from build123d import *

# Parameters (mm, degrees)
SKETCH1_W           = 40
SKETCH1_H           = 40
SKETCH1_W_2         = 36
SKETCH1_H_2         = 36
BOSS_EXTRUDE1_DEPTH = 1116
FILLET1_R           = 2
FILLET2_R           = 4


with BuildPart() as part:
    # Sketch1 → Boss-Extrude1 (new body)
    with BuildSketch(Plane.XY):
        Rectangle(SKETCH1_W, SKETCH1_H)
        Rectangle(SKETCH1_W_2, SKETCH1_H_2, mode=Mode.SUBTRACT)
    extrude(amount=BOSS_EXTRUDE1_DEPTH)

    # Fillet1
    fillet1_edges = [part.edges().sort_by_distance(p)[0] for p in [
        (18, -18, 558),
        (18, 18, 558),
        (-18, 18, 558),
        (-18, -18, 558),
    ]]
    fillet(fillet1_edges, radius=FILLET1_R)

    # Fillet2
    fillet2_edges = [part.edges().sort_by_distance(p)[0] for p in [
        (20, -20, 558),
        (-20, -20, 558),
        (-20, 20, 558),
        (20, 20, 558),
    ]]
    fillet(fillet2_edges, radius=FILLET2_R)


solid = part.part
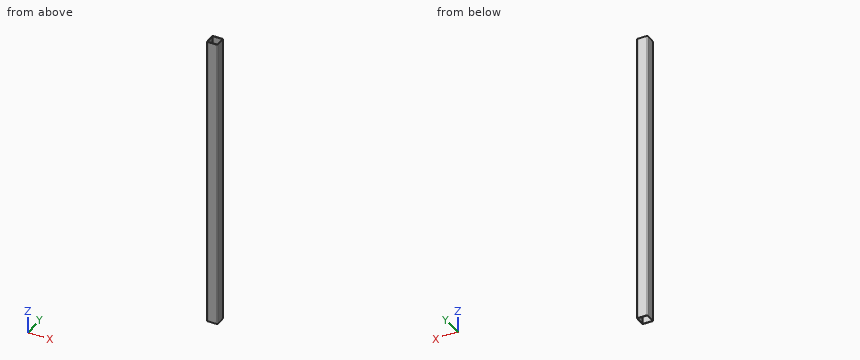
Verification items for the finished model (mm, model axes). Coordinates: 2 decimals unless noted, no trailing zeros. Write each loop counter-clockwise with the first axis right and the second up, starting at its lowest first coordinate (ties: lowest second). Pieces come first, ordered by that corner, then holes. Notation, with made-up numbers: M -22,-23 L 35,-23 A20 ccw 35,-3 Z; hole C 51.5,10.5 d4. An arc over 180 degrees is marked long. Use a Markdown table: item, result.
Q1. Sectioned sample at C-C, the plane z = 978. Record the boundary of the cut face in (x, y).
Reply:
| item | result |
|---|---|
| outline | M -20,-16 A4 ccw -16,-20 L 16,-20 A4 ccw 20,-16 L 20,16 A4 ccw 16,20 L -16,20 A4 ccw -20,16 Z; hole M -18,-16 A2 ccw -16,-18 L 16,-18 A2 ccw 18,-16 L 18,16 A2 ccw 16,18 L -16,18 A2 ccw -18,16 Z |
Q2. Sectioned sample at A-A, the plane x = -6.5. Record the boundary of the cut face in (y, z).
Reply:
| item | result |
|---|---|
| outline | M -20,0 L -18,0 L -18,1116 L -20,1116 Z; M 18,0 L 20,0 L 20,1116 L 18,1116 Z |
Q3. Thickness scan on line 1 (Y direction, x = 10, z = 511.5); line 2 (Y direction, x = -17.5, z = 381.5). Record the ranges inside material, lowest first.
Reply:
| item | result |
|---|---|
| line 1 | y = -20 to -18, 18 to 20 |
| line 2 | y = -19.71 to -17.32, 17.32 to 19.71 |
Q4. Go/stop test with a flat-tipped pin: P1, Ø12, axis at x = 15.5, y = 4.5, coming from the +Z side. Record where the tip stops, or that it passes through.
Reply:
| item | result |
|---|---|
| P1 | stops at z = 1116 |
